```python
from build123d import *

# Parameters (mm, degrees)
SKETCH1_R                 = 40
SKETCH1_R_2               = 16
BOSS_EXTRUDE1_DEPTH       = 16
SKETCH2_R                 = 21
CUT_EXTRUDE1_DEPTH        = 10
M10_CLEARANCE_HOLE1_D     = 11
M10_CLEARANCE_HOLE1_DEPTH = 29.25
M10_CLEARANCE_HOLE1_TIP   = 3.304733405


with BuildPart() as part:
    # Sketch1 → Boss-Extrude1 (new body)
    with BuildSketch(Plane(origin=(0, 0, 0), x_dir=(1, 0, 0), z_dir=(0, 1, 0))):
        with Locations(Location((0, 0, 0), (0, 0, 270))):
            Circle(SKETCH1_R)
        with Locations(Location((0, 0, 0), (0, 0, 270))):
            Circle(SKETCH1_R_2, mode=Mode.SUBTRACT)
    extrude(amount=BOSS_EXTRUDE1_DEPTH)

    # Sketch2 → Cut-Extrude1 (cut)
    with BuildSketch(Plane(origin=(0, 16, 0), x_dir=(1, 0, 0), z_dir=(0, 1, 0))):
        with Locations(Location((0, 0, 0), (0, 0, 270))):
            Circle(SKETCH2_R)
    extrude(amount=-CUT_EXTRUDE1_DEPTH, mode=Mode.SUBTRACT)

    # M10 Clearance Hole1
    with Locations(Plane(origin=(0, 16, 0), x_dir=(1, 0, 0), z_dir=(0, 1, 0))):
        with Locations((0, -30), (0, 30), (-30, 0), (30, 0)):
            Hole(M10_CLEARANCE_HOLE1_D / 2, depth=M10_CLEARANCE_HOLE1_DEPTH)
            with Locations((0, 0, -(M10_CLEARANCE_HOLE1_DEPTH + M10_CLEARANCE_HOLE1_TIP / 2))):  # 118° drill point
                Cone(0, M10_CLEARANCE_HOLE1_D / 2, M10_CLEARANCE_HOLE1_TIP, mode=Mode.SUBTRACT)


solid = part.part
```
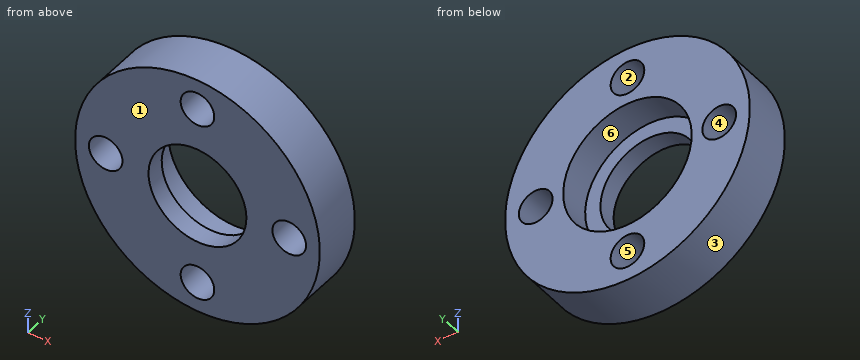
The listing builds one solid part. Answer for the finished solid, in the listing's coordinates (mm). Face numbers are marked on the shaded views. A direction names the side the tool comes from. Coordinates: 2 decimals unless noted, no trailing zeros. Loops run counter-clockwise (first coordinate to the right, second up) from the corner with the lowest first, then second, coordinate; pieces in that order, holes last. Notation, with made-up numbers: M 1.25,-27.75 L 6.25,-27.75 A19 ccw 6.25,-18.75 Z; hole C 71.5,68 d7. An arc over 180 degrees is marked long. Answer as a JSON object with one key per item and string values. Group by question number.
Item 1: Consider L1, parallel to Z at x = -0.5, y = 6.5; L2, parallel to Z at x = 4, y = 8.75; L3, parallel to X at y = 9.5, z = 1. Determine where each line is inside the solid, lowest interval first.
Item 2: Section C-C (x = 26.5) is taken. Write down the section's boundary in (y, z), and give its area (3 significant figures).
Item 3: Section B-B (y = 11.5) is taken. Write down the section's boundary in (x, z), and give its area (3 significant figures).
Item 4: Section D-D (z = 28.5) is taken. Write down the section's boundary in (x, y).
Item 5: Determine the mould class of the marked faces 1, 2, 3 and 4 for opening direction X: +X half, -X half, draft (parallel to the pull), parting line (faces both ways), or undercut.
Item 6: Which of the six approach directions +Z, -Z, +X, -X, +Y, -Y give full straight-line access (tool end or side, diameter ignored) to the marked faces 5 and 6?
Item 7: Section A-A (z = 0) is taken. Write down the section's boundary in (x, y), and give its area (3 significant figures).
Item 8: Each of these flat-tipped pins is pushed along its axis until it touches: P1, Ø8, axis at x = -15, z = -13, coming from the +Y side; P2, Ø3, axis at y = 10, z = 8, coming from the +X side; P3, Ø8, axis at y = 11, z = -13.5, coming from the +X side; P4, Ø5, axis at x = -27, y = 3, coming from the +Z side. Where does it stop, or does it pass through?
Solved:
{
 "1": {"L1": "z = -40 to -35.48, -24.52 to -20.99, 20.99 to 24.52, 35.48 to 40", "L2": "z = -39.8 to -33.77, -26.23 to -20.62, 20.62 to 26.23, 33.77 to 39.8", "L3": "x = -39.99 to -35.41, -24.59 to -20.98, 20.98 to 24.59, 35.41 to 39.99"},
 "2": {"outline": "M 0,-29.96 L 16,-29.96 L 16,-4.24 L 0,-4.24 Z; M 0,4.24 L 16,4.24 L 16,29.96 L 0,29.96 Z", "area": "823 mm2"},
 "3": {"outline": "C 0,0 d80; hole C -30,0 d11; hole C 0,0 d42; hole C 0,-30 d11; hole C 0,30 d11; hole C 30,0 d11", "area": "3,260 mm2"},
 "4": {"outline": "M -28.07,0 L -5.29,0 L -5.29,16 L -28.07,16 Z; M 5.29,0 L 28.07,0 L 28.07,16 L 5.29,16 Z"},
 "5": {"face 1": "draft", "face 2": "undercut", "face 3": "parting line", "face 4": "undercut"},
 "6": {"face 5": "+Y, -Y", "face 6": "+Y"},
 "7": {"outline": "M -40,0 L -35.5,0 L -35.5,16 L -40,16 Z; M -24.5,0 L -16,0 L -16,6 L -21,6 L -21,16 L -24.5,16 Z; M 16,0 L 24.5,0 L 24.5,16 L 21,16 L 21,6 L 16,6 Z; M 35.5,0 L 40,0 L 40,16 L 35.5,16 Z", "area": "316 mm2"},
 "8": {"P1": "stops at y = 16", "P2": "stops at x = 39.47", "P3": "stops at x = 38.86", "P4": "stops at z = 31.62"}
}
